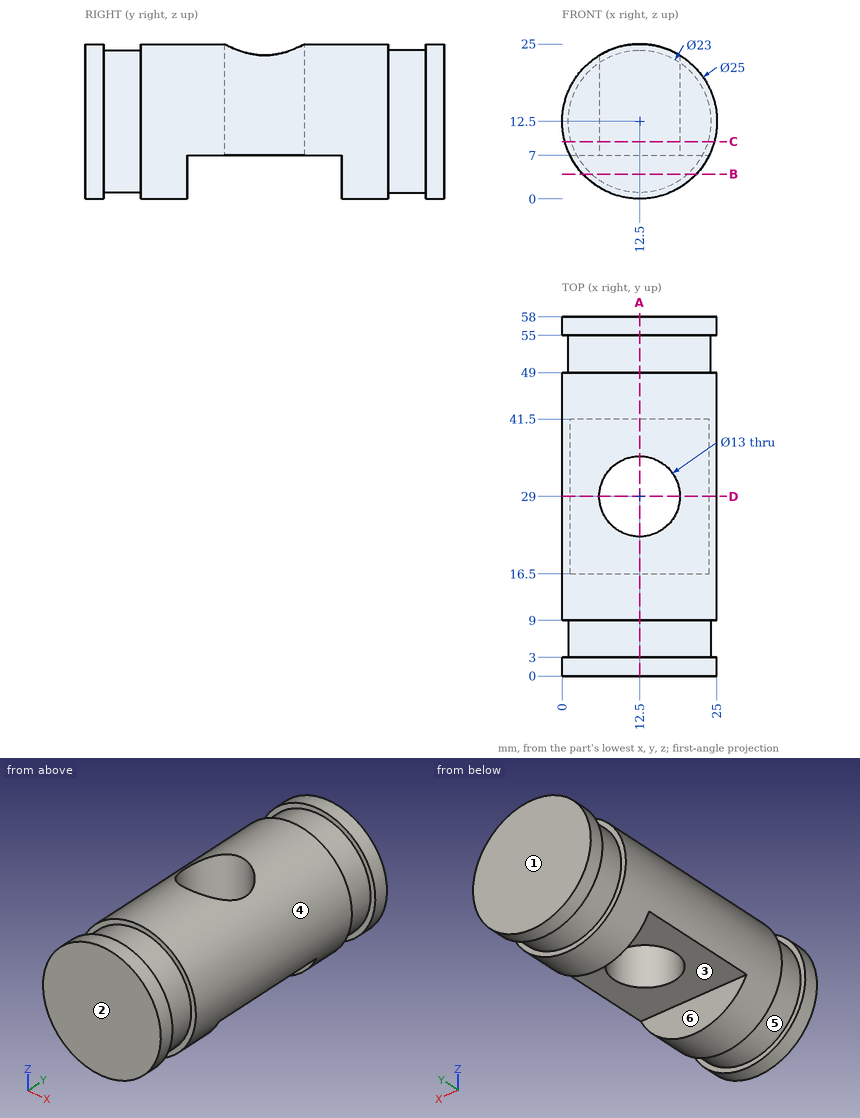
Design review of the part shown in the three views and the two pictorial views. Dimensions are in mm from the part's minimum x, y and z. A direction names the side the tool comes from. Coordinates: 2 decimals unless noted, no trailing zeros. Write each loop counter-clockwise with the first axis right and the second up, starting at its lowest first coordinate (ties: lowest second). Pieces come first, ordered by that corner, then holes. Notation, with made-up numbers: (88.25, 70) - (106.25, 70) arc R27 cw to (106.25, 106) - close; hole circle Ø6 at (42, 61). An arc over 180 degrees is marked (long way). Write item = value, one per line.
(1) Consider section D-D, the plane y = 29. Give the boundary of the cut face in (x, z).
Result sheet:
outline = (1.28, 7) - (6, 7) - (6, 23.18) arc R12.5 ccw to start; (19, 7) - (23.72, 7) arc R12.5 ccw to (19, 23.18) - close
(2) For P1, Ø11, axis at x = 14.5, y = 32, coming from the -Z side; P2, Ø12, axis at x = 21.5, y = 20, coming from the +Z side; P3, Ø2, axis at x = 15.5, y = 20.5, coming from the +Z side, all flat-tipped, find the tip position at first contact; note any pin that passes through.
Result sheet:
P1 = 7
P2 = 24.63
P3 = 24.84
(3) Consider section A-A, the plane x = 12.5. Give the boundary of the cut face in (y, z).
Result sheet:
outline = (0, 0) - (3, 0) - (3, 1) - (9, 1) - (9, 0) - (16.5, 0) - (16.5, 7) - (22.5, 7) - (22.5, 25) - (9, 25) - (9, 24) - (3, 24) - (3, 25) - (0, 25) - close; (35.5, 7) - (41.5, 7) - (41.5, 0) - (49, 0) - (49, 1) - (55, 1) - (55, 0) - (58, 0) - (58, 25) - (55, 25) - (55, 24) - (49, 24) - (49, 25) - (35.5, 25) - close
(4) For line 1 (Y direction, x = 8.75, z = 3.5); line 2 (Z direction, x = 12, y = 39.5); line 3 (Y direction, x = 13.5, z = 21.5), list the stretches that pass through material, from the lowest coordinate up. Write a range as [from, to].
Result sheet:
line_1 = [0, 16.5], [41.5, 58]
line_2 = [7, 24.99]
line_3 = [0, 22.58], [35.42, 58]
(5) Mouldability with a two-part tool opening along Y and no side actions: class the marked faces 1, 2 and 3 as pulls with the +Y half, pulls with the -Y half, needs draft (parallel to the pull), parting line crosses it, or undercut.
Result sheet:
face_1 = pulls with the +Y half
face_2 = pulls with the -Y half
face_3 = undercut
(6) Consider section C-C, the plane z = 9.25. Give the boundary of the cut face in (x, y), then the cut area to 3 significant figures.
Result sheet:
outline = (0.43, 0) - (24.57, 0) - (24.57, 3) - (23.53, 3) - (23.53, 9) - (24.57, 9) - (24.57, 49) - (23.53, 49) - (23.53, 55) - (24.57, 55) - (24.57, 58) - (0.43, 58) - (0.43, 55) - (1.47, 55) - (1.47, 49) - (0.43, 49) - (0.43, 9) - (1.47, 9) - (1.47, 3) - (0.43, 3) - close; hole circle Ø13 at (12.5, 29)
area = 1,240 mm^2
(7) Consider section B-B, the plane z = 4. Give the boundary of the cut face in (x, y), then the cut area to 3 significant figures.
Result sheet:
outline = (3.33, 0) - (21.67, 0) - (21.67, 3) - (20.25, 3) - (20.25, 9) - (21.67, 9) - (21.67, 16.5) - (3.33, 16.5) - (3.33, 9) - (4.75, 9) - (4.75, 3) - (3.33, 3) - close; (3.33, 41.5) - (21.67, 41.5) - (21.67, 49) - (20.25, 49) - (20.25, 55) - (21.67, 55) - (21.67, 58) - (3.33, 58) - (3.33, 55) - (4.75, 55) - (4.75, 49) - (3.33, 49) - close
area = 571 mm^2
(8) Machinability: for the marked faces 4, 5 and 6, which of the approach directions +Z, -Z, +X, -X, +Y, -Y give a long, thin tool a straight path to every point of the face, cutting with its end or side? Answer none if there is none.
Result sheet:
face_4 = +Y, -Y
face_5 = none
face_6 = -Z, +X, -X
